Input: dimensioned drawing with shaded views. Units: mm. Origin: part minimum x, y, z. Give positions to 0.01 mm unless a question says otherwise; leave off trailing zeros. Write each loop counter-clockwise with the first axis right and the second up, starting at its lowest first coordinate (ties: lowest second). Pieces come first, ordered by that corner, then holes. Notation, with made-up numbers: (0.25, -34) -> (24.25, -34) arc R15 ccw to (24.25, -21) -> close; hole circle Ø5 at (54.25, 51.25). An arc over 180 degrees is marked (long way). Answer as a JSON object with one key per item and string values. Group by question number.
(1) Section query D-D on y = 226.5. Output: boundary loops of the cut face in (x, z).
(2) Contact query for flat-ended pins moving along their axis: pin 1 Ø1.5 at (x, z) = (144.5, 26.5) entering from -Y; pin 2 Ø3 at (y, z) = (179.5, 13.5) entering from -X; pin 3 Ø1.7 at (x, z) = (96.5, 26) entering from -Y. Output: stop coordinate, or through.
(3) Section query C-C on x = 136. Output: boundary loops of the cut face in (y, z).
(4) Section query A-A on y = 163. Output: boundary loops of the cut face in (x, z), plus the area to 3 significant figures.
(5) Draft query along X for the marked faces 1 and 2. Return one class per face: +X half, -X half, draft (parallel to the pull), parting line (faces both ways), or undercut.
(6) Material intervals for probe 1 along X at (y, z) = (80, 21); probe 2 along Z at (x, y) = (80, 328); probe 3 along Y at (x, z) = (138, 13.5), sorted ascending.
(7) Section query B-B on z = 5.5. Output: boundary loops of the cut face in (x, y), plus the area to 3 significant figures.
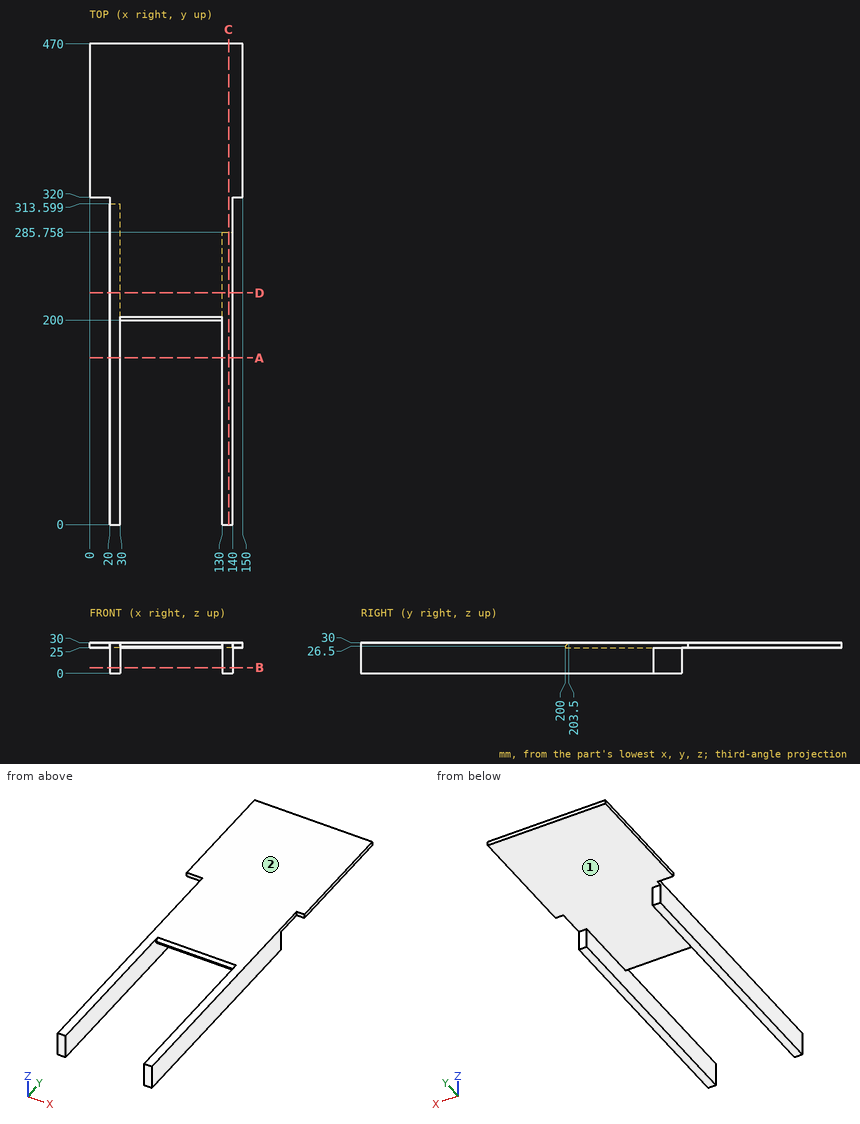
Answer list:
{
 "1": {"outline": "(20, 0) -> (30, 0) -> (30, 25) -> (130, 25) -> (130, 0) -> (140, 0) -> (140, 30) -> (20, 30) -> close"},
 "2": {"pin 1": "y = 320", "pin 2": "x = 20", "pin 3": "y = 200"},
 "3": {"outline": "(0, 0) -> (285.76, 0) -> (285.76, 25) -> (470, 25) -> (470, 30) -> (0, 30) -> close"},
 "4": {"outline": "(20, 0) -> (30, 0) -> (30, 30) -> (20, 30) -> close; (130, 0) -> (140, 0) -> (140, 30) -> (130, 30) -> close", "area": "600 mm2"},
 "5": {"face 1": "undercut", "face 2": "draft"},
 "6": {"probe 1": "20 to 30, 130 to 140", "probe 2": "25 to 30", "probe 3": "0 to 285.76"},
 "7": {"outline": "(20, 0) -> (30, 0) -> (30, 313.6) -> (20, 313.6) -> close; (130, 0) -> (140, 0) -> (140, 285.76) -> (130, 285.76) -> close", "area": "5,990 mm2"}
}
